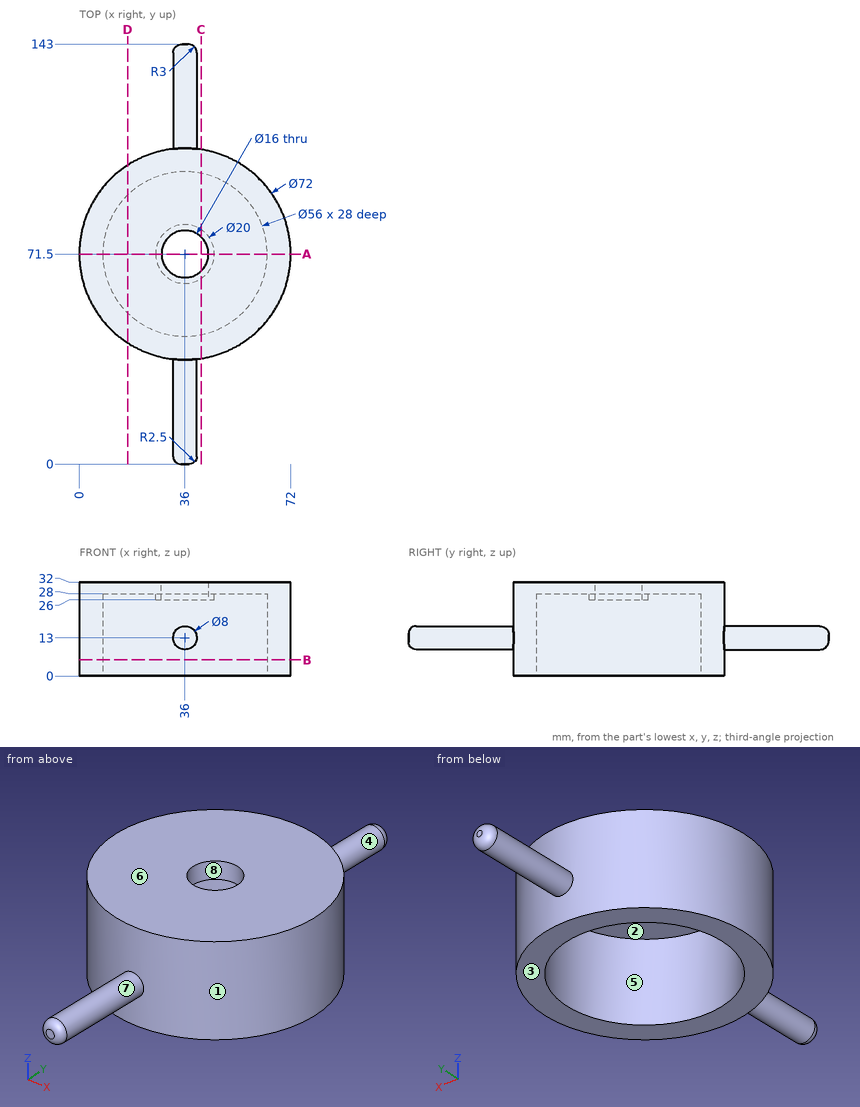
For this review, use the dimensioned drawing (mm, ordinates from the lowest corner) and the shaded views. A direction names the side the tool comes from. Round coordinates to 2 decimals unless told otherwise and drop trailing zeros. Order: outer loops, then holes, each group sorted by start corner. A loop starts at its lowest first (then second) coordinate and runs counter-clockwise, first axis right, second up. Notation, with made-up numbers: (86, 69) - (106, 69) arc R22 cw to (106, 103) - close; hole circle Ø6 at (-23, 54.5). An arc over 180 degrees is marked (long way). Use one line per item in the form item = value.
Q1. Add section A-A on y = 71.5. Give the boundary of the cut face in (x, z), then the cut area to 3 significant figures.
Response values:
outline = (0, 0) - (8, 0) - (8, 28) - (26, 28) - (26, 26) - (28, 26) - (28, 32) - (0, 32) - close; (44, 26) - (46, 26) - (46, 28) - (64, 28) - (64, 0) - (72, 0) - (72, 32) - (44, 32) - close
area = 680 mm^2
Q2. Tool access review of the marked faces 4, 5, 6, 7 and 8: name each direction out of +Z, -Z, +X, -X, +Y, -Y from which nothing blocks a thin tool from reaching the whole face with its end or side.
Response values:
face_4 = +Y
face_5 = -Z
face_6 = +Z, +X, -X, +Y, -Y
face_7 = -Y
face_8 = +Z, -Z
Q3. Add section D-D on x = 16.5. Give the boundary of the cut face in (y, z), then the cut area to 3 significant figures.
Response values:
outline = (41.24, 0) - (51.41, 0) - (51.41, 28) - (91.59, 28) - (91.59, 0) - (101.76, 0) - (101.76, 32) - (41.24, 32) - close
area = 811 mm^2
Q4. Add section C-C on x = 41.5. Give the boundary of the cut face in (y, z), then the cut area to 3 significant figures.
Response values:
outline = (35.92, 0) - (44.05, 0) - (44.05, 28) - (63.15, 28) - (63.15, 26) - (65.69, 26) - (65.69, 32) - (35.92, 32) - close; (77.31, 26) - (79.85, 26) - (79.85, 28) - (98.95, 28) - (98.95, 0) - (107.08, 0) - (107.08, 32) - (77.31, 32) - close
area = 703 mm^2
Q5. Add section B-B on z = 5.5. Give the boundary of the cut face in (x, y).
Response values:
outline = circle Ø72 at (36, 71.5); hole circle Ø56 at (36, 71.5)
Q6. To check wall thickness, follow line 1 (Y direction, x = 36, z = 28.85); line 2 (Y direction, x = 36, z = 7); line 3 (X direction, y = 71, z = 6). State the ranges of each line that lie inside material, in increasing order.
Response values:
line_1 = 35.5 to 63.5, 79.5 to 107.5
line_2 = 35.5 to 43.5, 99.5 to 107.5
line_3 = 0 to 8, 64 to 72
Q7. Mouldability with a two-part tool opening along X and no side actions: class the marked faces 1, 2 and 3 as pulls with the +X half, pulls with the -X half, needs draft (parallel to the pull), parting line crosses it, or undercut.
Response values:
face_1 = parting line crosses it
face_2 = undercut
face_3 = needs draft
Q8. Clearance check with flat-ended pins moving along their axes: P1, Ø10, axis at x = 50.5, z = 26, coming from the +Y side; P2, Ø1, axis at x = 9.5, z = 24.5, coming from the +Y side; P3, Ø6, axis at y = 36.5, z = 8.5, coming from the -X side; P4, Ø8, axis at y = 29.5, z = 28.5, coming from the +X side. State where each tip first meets the part, or that it passes through.
Response values:
P1 = 106.22
P2 = 96.4
P3 = 19.51
P4 = through
